from build123d import *

# Parameters (mm, degrees)
CUT_EXTRUDE_1_DEPTH  = 169.169557293
SKETCH_4_OUTSIDE_W   = 262.768
SKETCH_4_OUTSIDE_H   = 262.768
SKETCH_4_OUTSIDE_W_2 = 192
SKETCH_4_OUTSIDE_H_2 = 141
CUT_EXTRUDE_2_DEPTH  = 169.169557293


with BuildPart() as part:
    # 草图1 → 旋转1 (revolve)
    with BuildSketch(Plane(origin=(0, 0, 0), x_dir=(1, 0, 0), z_dir=(0, 1, 0))):
        Polygon((0, 111), (-7.5, 111), (-7.5, 106), (-7.15, 106), (-7.15, 104.9), (-7.5, 104.9), (-7.5, 60), (-10, 60), (-10, 55), (-30, 55), (-30, 20), (-100, 20), (-100, 0), (0, 0), align=None)
    revolve(axis=Axis((0, 0, 0), (0, 0, 1)))

    # 草图3 → 切除-拉伸1 (cut, through all)
    with BuildSketch(Plane(origin=(0, 0, -20), x_dir=(-1, 0, 0), z_dir=(0, 0, -1))):
        with BuildLine():
            Line((-20, 55.5), (20, 55.5))
            ThreePointArc((20, 55.5), (25.5, 50), (20, 44.5))
            Line((20, 44.5), (-20, 44.5))
            ThreePointArc((-20, 44.5), (-25.5, 50), (-20, 55.5))
        make_face()
        with BuildLine():
            Line((-40.5, -5.5), (-80.5, -5.5))
            ThreePointArc((-80.5, -5.5), (-86, 0), (-80.5, 5.5))
            Line((-80.5, 5.5), (-40.5, 5.5))
            ThreePointArc((-40.5, 5.5), (-35, 0), (-40.5, -5.5))
        make_face()
    cut_extrude_1 = extrude(amount=-CUT_EXTRUDE_1_DEPTH, mode=Mode.SUBTRACT)

    # 镜向1: 切除-拉伸1 across plane
    add(cut_extrude_1.mirror(Plane(origin=(0, 0, 0), x_dir=(0, 0, 1), z_dir=(1, 0, 0))), mode=Mode.SUBTRACT)

    # 镜向2: 切除-拉伸1 across plane
    add(cut_extrude_1.mirror(Plane.ZX), mode=Mode.SUBTRACT)

    # 草图4 outside → 切除-拉伸2 (cut, through all)
    with BuildSketch(Plane(origin=(0, 0, -20), x_dir=(-1, 0, 0), z_dir=(0, 0, -1))):
        Rectangle(SKETCH_4_OUTSIDE_W, SKETCH_4_OUTSIDE_H)
        Rectangle(SKETCH_4_OUTSIDE_W_2, SKETCH_4_OUTSIDE_H_2, mode=Mode.SUBTRACT)
    extrude(amount=-CUT_EXTRUDE_2_DEPTH, mode=Mode.SUBTRACT)


solid = part.part
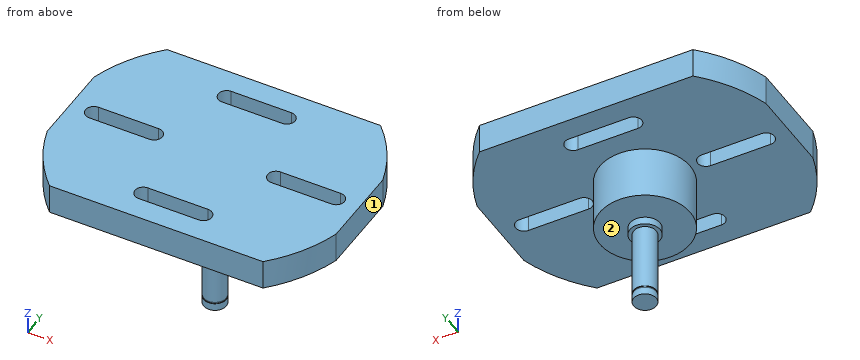
The listing builds one solid part. Answer for the finished solid, in the listing's coordinates (mm). Face numbers are marked on the shaded views. A direction names the side the tool comes from. Coordinates: 2 decimals unless noted, no trailing zeros. Write each loop counter-clockwise with the first axis right and the second up, starting at its lowest first coordinate (ties: lowest second). Pieces come first, ordered by that corner, then holes. Notation, with made-up numbers: M 35.5,13 L 90.5,13 A17 cw 90.5,34 Z; hole C 44.25,89.5 d4. An arc over 180 degrees is marked long. Put each result on its own line as item: value. Start each with the question number.
1. A flat-ended cylindrical pin translates along its axis: P1, Ø3, axis at x = 24, y = -41, coming from the -Z side. Find the tip coordinate at first contact, or state that the pin passes through.
2. Consider line 1 (Z direction, x = -65, y = -15.5); line 2 (X direction, y = 1, z = -31.5); line 3 (Z direction, x = 4, y = 17). Determine where each line is inside the solid, lowest interval first. Write a range as from..to.
3. A cutting plane is placed at A-A on x = 57. Write down the section's boundary in (y, z).
4. A cutting plane is placed at B-B on y = 0. Count the separate pieces of the cut face and the enclosed holes in it, then the cut area to 3 significant figures.
5. A cutting plane is placed at D-D on z = -14.5. Write down the section's boundary in (x, y), then the cut area to 3 significant figures.
6. Which of the six approach directions +Z, -Z, +X, -X, +Y, -Y give full straight-line access (tool end or side, diameter ignored) to the marked faces 1 and 2?
Resolved:
1. P1: stops at z = -20
2. line 1: z = -20..0
2. line 2: x = -29.98..29.98
2. line 3: z = -55..0
3. outline: M -70.5,-20 L -5.5,-20 L -5.5,0 L -70.5,0 Z; M 5.5,-20 L 70.5,-20 L 70.5,0 L 5.5,0 Z
4. separate pieces: 3
4. enclosed holes: 0
4. area: 4,760 mm2
5. outline: M -96,-28 A100 ccw -70.92,-70.5 L 70.92,-70.5 A100 ccw 96,-28 L 96,28 A100 ccw 70.92,70.5 L -70.92,70.5 A100 ccw -96,28 Z; hole M -80.5,-5.5 L -40.5,-5.5 A5.5 ccw -40.5,5.5 L -80.5,5.5 A5.5 ccw Z; hole M -20,-55.5 L 20,-55.5 A5.5 ccw 20,-44.5 L -20,-44.5 A5.5 ccw Z; hole M -20,44.5 L 20,44.5 A5.5 ccw 20,55.5 L -20,55.5 A5.5 ccw Z; hole M 40.5,-5.5 L 80.5,-5.5 A5.5 ccw 80.5,5.5 L 40.5,5.5 A5.5 ccw Z
5. area: 23,200 mm2
6. face 1: +Z, -Z, +X, +Y, -Y
6. face 2: -Z
